Work out the finished part from the listing and answer in its coordinate system (mm). A direction names the side the tool comes from. Coordinates: 2 decimals unless noted, no trailing zeros. Order: outer loops, then holes, each group sorted by start corner. A loop starts at its lowest first (then second) coordinate and runs counter-clockwise, first axis right, second up. Notation, with made-up numbers: M 47,25 L 90,25 A13 cw 90,33 Z; hole C 16.5,13 d1. An arc over 180 degrees is marked long. Answer in a Markdown table with one row per item. Add a question column.
Item 1: The part is cut by section B-B (y = 14.5). Write down the section's boundary in (x, z).
Item 2: Which of the six approach directions +Z, -Z, +X, -X, +Y, -Y give full straight-line access (tool end or side, diameter ignored) to faces 5 (the face through (0, 16.25, 2)), 6 (the face through (15.14, 21.6, 4.06)), 7 (the face through (0, -17.5, 6))?
Item 3: The part is cut by section A-A (x = 1.5). Write down the section's boundary in (y, z), then the cut area to 4 significant figures.
Item 4: The mould has two halves that part along Y. Classify faces 1 (the face through (0, 12.75, 2)), 2 (the face through (0, 0, 0)), 3 (the face through (0, -12.75, 2)), 4 (the face through (-15.14, 21.6, 4.06)): released by +Y, released by -Y, zero draft, split by the parting line, or undercut.
Item 5: The part is cut by section C-C (z = 4). Write down the section's boundary in (x, y), then the cut area to 3 significant figures.
Item 6: The part is cut by section D-D (y = -12). Write down the section's boundary in (x, z), then the cut area to 3 significant figures.
Item 7: Flat-ended cylindrical pins translate along their axes: pin 1 Ø10 at (x, y) = (-7.5, -5) entering from -Z; pin 2 Ø1.8 at (x, y) = (-1, -14.5) entering from +Z. Find the tip coordinate at first contact, or state that the pin passes through.
Item 8: Consider line 1 (Y direction, x = -3.5, z = 7); line 2 (Y direction, x = 0.5, z = 3.75); line 3 (X direction, y = 12, z = 5). Determine where each line is inside the solid, lowest interval first. Write a range as from..to.
from build123d import *

# Parameters (mm, degrees)
SKETCH1_W           = 32
SKETCH1_H           = 45
BOSS_EXTRUDE1_DEPTH = 8
FILLET1_R           = 3
CUT_EXTRUDE1_DEPTH  = 29.744564704
CUT_EXTRUDE2_DEPTH  = 3.3


with BuildPart() as part:
    # Sketch1 → Boss-Extrude1 (new body)
    with BuildSketch(Plane.XY):
        Rectangle(SKETCH1_W, SKETCH1_H)
    extrude(amount=BOSS_EXTRUDE1_DEPTH)

    # Fillet1
    fillet1_edges = [part.edges().sort_by_distance(p)[0] for p in [
        (-16, 22.5, 4),
        (16, 22.5, 4),
        (16, -22.5, 4),
        (-16, -22.5, 4),
    ]]
    fillet(fillet1_edges, radius=FILLET1_R)

    # Sketch2 → Cut-Extrude1 (cut, through all)
    with BuildSketch(Plane.XY.offset(8)):
        with BuildLine():
            Line((-5, 16.25), (5, 16.25))
            ThreePointArc((5, 16.25), (6.75, 14.5), (5, 12.75))
            Line((5, 12.75), (-5, 12.75))
            ThreePointArc((-5, 12.75), (-6.75, 14.5), (-5, 16.25))
        make_face()
        with BuildLine():
            Line((-5, -12.75), (5, -12.75))
            ThreePointArc((5, -12.75), (6.75, -14.5), (5, -16.25))
            Line((5, -16.25), (-5, -16.25))
            ThreePointArc((-5, -16.25), (-6.75, -14.5), (-5, -12.75))
        make_face()
    extrude(amount=-CUT_EXTRUDE1_DEPTH, mode=Mode.SUBTRACT)

    # Sketch3 → Cut-Extrude2 (cut)
    with BuildSketch(Plane.XY.offset(8)):
        with BuildLine():
            Line((-5, 17.5), (5, 17.5))
            ThreePointArc((5, 17.5), (8, 14.5), (5, 11.5))
            Line((5, 11.5), (-5, 11.5))
            ThreePointArc((-5, 11.5), (-8, 14.5), (-5, 17.5))
        make_face()
        with BuildLine():
            Line((-5, -11.5), (5, -11.5))
            ThreePointArc((5, -11.5), (8, -14.5), (5, -17.5))
            Line((5, -17.5), (-5, -17.5))
            ThreePointArc((-5, -17.5), (-8, -14.5), (-5, -11.5))
        make_face()
    extrude(amount=-CUT_EXTRUDE2_DEPTH, mode=Mode.SUBTRACT)


solid = part.part
Reply:
| question | item | result |
|---|---|---|
| 1 | outline | M -16,0 L -6.75,0 L -6.75,4.7 L -8,4.7 L -8,8 L -16,8 Z; M 6.75,0 L 16,0 L 16,8 L 8,8 L 8,4.7 L 6.75,4.7 Z |
| 2 | face 5 | +Z, -Z |
| 2 | face 6 | +Z, -Z, +X, +Y |
| 2 | face 7 | +Z |
| 3 | outline | M -22.5,0 L -16.25,0 L -16.25,4.7 L -17.5,4.7 L -17.5,8 L -22.5,8 Z; M -12.75,0 L 12.75,0 L 12.75,4.7 L 11.5,4.7 L 11.5,8 L -11.5,8 L -11.5,4.7 L -12.75,4.7 Z; M 16.25,0 L 22.5,0 L 22.5,8 L 17.5,8 L 17.5,4.7 L 16.25,4.7 Z |
| 3 | area | 287.5 mm2 |
| 4 | face 1 | undercut |
| 4 | face 2 | zero draft |
| 4 | face 3 | undercut |
| 4 | face 4 | released by +Y |
| 5 | outline | M -16,-19.5 A3 ccw -13,-22.5 L 13,-22.5 A3 ccw 16,-19.5 L 16,19.5 A3 ccw 13,22.5 L -13,22.5 A3 ccw -16,19.5 Z; hole M -5,-16.25 L 5,-16.25 A1.75 ccw 5,-12.75 L -5,-12.75 A1.75 ccw Z; hole M -5,12.75 L 5,12.75 A1.75 ccw 5,16.25 L -5,16.25 A1.75 ccw Z |
| 5 | area | 1,340 mm2 |
| 6 | outline | M -16,0 L 16,0 L 16,8 L 6.66,8 L 6.66,4.7 L -6.66,4.7 L -6.66,8 L -16,8 Z |
| 6 | area | 212 mm2 |
| 7 | pin 1 | stops at z = 0 |
| 7 | pin 2 | passes through |
| 8 | line 1 | y = -22.5..-17.5, -11.5..11.5, 17.5..22.5 |
| 8 | line 2 | y = -22.5..-16.25, -12.75..12.75, 16.25..22.5 |
| 8 | line 3 | x = -16..-6.66, 6.66..16 |
